Here's how the part is built. I have some questions about the finished solid (model axes, mm). A direction names the side the tool comes from. Round coordinates to 2 decimals unless told otherwise and drop trailing zeros. Order: outer loops, then holes, each group sorted by start corner. A loop starts at its lowest first (then second) coordinate and runs counter-clockwise, first axis right, second up.
```python
from build123d import *

# Parameters (mm, degrees)
SKETCH_1_R          = 7.5
EXTRUDE_1_DEPTH     = 24.5
SKETCH_2_OUTSIDE_W  = 27.678
SKETCH_2_OUTSIDE_H  = 27.678
SKETCH_2_OUTSIDE_R  = 4.9
CUT_EXTRUDE_1_DEPTH = 19
SKETCH_3_OUTSIDE_W  = 27.678
SKETCH_3_OUTSIDE_H  = 27.678
SKETCH_3_OUTSIDE_R  = 4
CUT_EXTRUDE_2_DEPTH = 10
SKETCH_4_OUTSIDE_W  = 27.678
SKETCH_4_OUTSIDE_H  = 27.678
SKETCH_4_OUTSIDE_R  = 5.9
CUT_EXTRUDE_3_DEPTH = 25
SKETCH_5_OUTSIDE_W  = 27.678
SKETCH_5_OUTSIDE_H  = 27.678
SKETCH_5_OUTSIDE_R  = 5
CUT_EXTRUDE_4_DEPTH = 15
CHAMFER_1_SIZE      = 0.5
SKETCH_6_W          = 15
SKETCH_6_H          = 6
CUT_EXTRUDE_5_DEPTH = 15


with BuildPart() as part:
    # 草图1 → 凸台-拉伸1 (new, symmetric)
    with BuildSketch(Plane.XY):
        Circle(SKETCH_1_R)
    extrude(amount=EXTRUDE_1_DEPTH, both=True)

    # 草图2 outside → 切除-拉伸1 (cut)
    with BuildSketch(Plane.XY.offset(24.5)):
        Rectangle(SKETCH_2_OUTSIDE_W, SKETCH_2_OUTSIDE_H)
        Circle(SKETCH_2_OUTSIDE_R, mode=Mode.SUBTRACT)
    extrude(amount=-CUT_EXTRUDE_1_DEPTH, mode=Mode.SUBTRACT)

    # 草图3 outside → 切除-拉伸2 (cut)
    with BuildSketch(Plane.XY.offset(24.5)):
        Rectangle(SKETCH_3_OUTSIDE_W, SKETCH_3_OUTSIDE_H)
        Circle(SKETCH_3_OUTSIDE_R, mode=Mode.SUBTRACT)
    extrude(amount=-CUT_EXTRUDE_2_DEPTH, mode=Mode.SUBTRACT)

    # 草图4 outside → 切除-拉伸3 (cut)
    with BuildSketch(Plane(origin=(0, 0, -24.5), x_dir=(-1, 0, 0), z_dir=(0, 0, -1))):
        Rectangle(SKETCH_4_OUTSIDE_W, SKETCH_4_OUTSIDE_H)
        Circle(SKETCH_4_OUTSIDE_R, mode=Mode.SUBTRACT)
    extrude(amount=-CUT_EXTRUDE_3_DEPTH, mode=Mode.SUBTRACT)

    # 草图5 outside → 切除-拉伸4 (cut)
    with BuildSketch(Plane(origin=(0, 0, -24.5), x_dir=(-1, 0, 0), z_dir=(0, 0, -1))):
        Rectangle(SKETCH_5_OUTSIDE_W, SKETCH_5_OUTSIDE_H)
        Circle(SKETCH_5_OUTSIDE_R, mode=Mode.SUBTRACT)
    extrude(amount=-CUT_EXTRUDE_4_DEPTH, mode=Mode.SUBTRACT)

    # 倒角1
    chamfer_1_edges = [part.edges().sort_by_distance(p)[0] for p in [
        (-4, 0, 24.5),
        (-7.5, 0, 0.5),
        (5, 0, -24.5),
        (-7.5, 0, 5.5),
    ]]
    chamfer(chamfer_1_edges, length=CHAMFER_1_SIZE)

    # 草图6 → 切除-拉伸5 (cut)
    with BuildSketch(Plane.XY.offset(5.5)):
        with Locations((0, 9.9)):
            Rectangle(SKETCH_6_W, SKETCH_6_H)
        with Locations((0, -9.9)):
            Rectangle(SKETCH_6_W, SKETCH_6_H)
    extrude(amount=-CUT_EXTRUDE_5_DEPTH, mode=Mode.SUBTRACT)


solid = part.part
```
1. If we section it at B-B, the plane x = 0: Write out the boundary of the cut face in (y, z), and give its area (3 significant figures).
Evaluation:
outline: (-6.9, 0.5) - (-5.9, 0.5) - (-5.9, -9.5) - (-5, -9.5) - (-5, -24) - (-4.5, -24.5) - (4.5, -24.5) - (5, -24) - (5, -9.5) - (5.9, -9.5) - (5.9, 0.5) - (6.9, 0.5) - (6.9, 5.5) - (4.9, 5.5) - (4.9, 14.5) - (4, 14.5) - (4, 24) - (3.5, 24.5) - (-3.5, 24.5) - (-4, 24) - (-4, 14.5) - (-4.9, 14.5) - (-4.9, 5.5) - (-6.9, 5.5) - close
area: 505 mm2
2. I need wall thicknesses on probe 1 along Z at (x, y) = (5.5, 1); probe 2 along X at (y, z) = (1, -17.5); probe 3 along Z at (x, y) = (-5.75, -1.75). Which ranges of each line are inside material? Lowest first, please.
Evaluation:
probe 1: z = -9.5 to 5.5
probe 2: x = -4.9 to 4.9
probe 3: z = 0.5 to 5.5
3. If we section it at C-C, the plane z = 18: Write out the boundary of the cut face in (x, y).
Evaluation:
outline: circle Ø8 at (0, 0)
4. I'm going to push flat-ended pins straight in: P1, Ø1, axis at y = 2.5, z = 10.5, coming from the -X side; P2, Ø3, axis at x = 4, z = -16.5, coming from the -Y side; P3, Ø1.5, axis at y = -0.5, z = -18.5, coming from the -X side. Where does each tip first touch, or does it pass through?
Evaluation:
P1: stops at x = -4.47
P2: stops at y = -4.33
P3: stops at x = -5
5. On a 3-axis mill with a long thin cutter (end or side, diameter ignored), from which of +Z, -Z, +X, -X, +Y, -Y can I reach the whole of each face in a straight line? I mean faces 1 (the cylindrical face through (-1.062, -4.783, 10.063)), 2 (the flat face through (5, -2, -9.5)), 3 (the conical face through (-7.134, 0.14, 5.365)). Say none if no direction works.
Evaluation:
face 1: +Z
face 2: -Z
face 3: +Z, -X
6. If we section it at A-A, the plane y = 0: Write out the boundary of the cut face in (x, z).
Evaluation:
outline: (-7.5, 1) - (-7, 0.5) - (-5.9, 0.5) - (-5.9, -9.5) - (-5, -9.5) - (-5, -24) - (-4.5, -24.5) - (4.5, -24.5) - (5, -24) - (5, -9.5) - (5.9, -9.5) - (5.9, 0.5) - (7, 0.5) - (7.5, 1) - (7.5, 5) - (7, 5.5) - (4.9, 5.5) - (4.9, 14.5) - (4, 14.5) - (4, 24) - (3.5, 24.5) - (-3.5, 24.5) - (-4, 24) - (-4, 14.5) - (-4.9, 14.5) - (-4.9, 5.5) - (-7, 5.5) - (-7.5, 5) - close
7. If we section it at D-D, the plane z = -18: Write out the boundary of the cut face in (x, y), and give its area (3 significant figures).
Evaluation:
outline: circle Ø10 at (0, 0)
area: 78.5 mm2
